```python
from build123d import *


with BuildPart() as part:
    # 扫描1: sweep along a path in 草图1
    with BuildLine(Plane(origin=(0, 0, 0), x_dir=(0, 0, -1), z_dir=(1, 0, 0))) as sweep_1_path:
        Line((9.103840683, 79.480312561), (356.051920341, 39.740156281))
        ThreePointArc((356.051920341, 39.740156281), (391.5, 0), (356.051920341, -39.740156281))
        Line((356.051920341, -39.740156281), (9.103840683, -79.480312561))
        ThreePointArc((9.103840683, -79.480312561), (-80, 0), (9.103840683, 79.480312561))
    # 草图2 → 扫描1 (sweep)
    with BuildSketch(Plane.XY):
        Polygon((-5, 80), (5, 80), (3.165615911, 74), (-3.165615911, 74), align=None)
    sweep(path=sweep_1_path.line)


solid = part.part
```
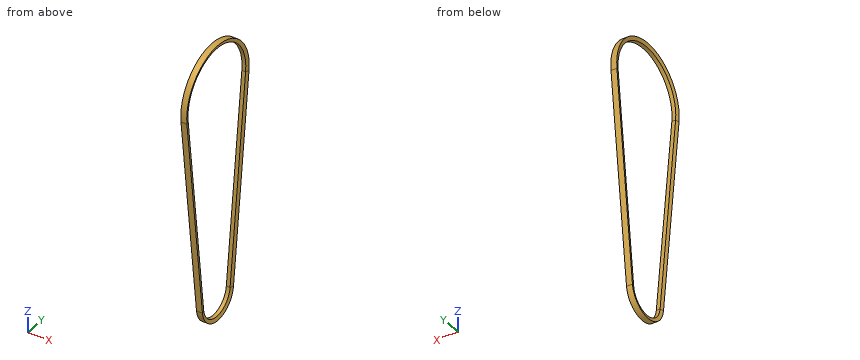
The model under review builds one solid part; all positions refer to its coordinate system, in mm. Coordinates: 2 decimals unless noted, no trailing zeros. Write each loop counter-clockwise with the first axis right and the second up, starting at its lowest first coordinate (ties: lowest second). Pieces come first, ordered by that corner, then holes. Notation, with made-up numbers: (16.5, 42) - (44.5, 42) arc R5 cw to (44.5, 48) - close; hole circle Ø5 at (57, 4). An arc over 180 degrees is marked (long way). Answer in a Markdown table with one row per item. Add a question column.
Q1. Consider section B-B on y = 0. Give the boundary of the cut face in (x, z), then the cut area to 3 significant figures.
Q2. Consider section C-C on x = 0.75. Give the boundary of the cut face in (y, z).
Q3. Clearance check with flat-ended pins moving along their axes: pin 1 (2 mm diameter, centred on x = 1, y = -33.5, fed in from -Z); pin 2 (12 mm diameter, centred on y = 47, z = -304, fed in from +X); pin 3 (1 mm diameter, centred on x = -1, y = 43.5, fed in from +Z). State where each tip first meets the part, or that it passes through.
Q4. Consider section A-A on z = 0. Give the boundary of the cut face in (x, y), then the cut area to 3 significant figures.
Q5. To check wall thickness, follow line 1 along Y through (x, z) = (-0.5, 0); line 2 along Z through (x, y) = (1.75, 0); line 3 along Y through (x, z) = (0.75, 30). State the ranges of each line that lie inside material, in increasing order. Write a range as from..to.
Answers below:
| question | item | result |
|---|---|---|
| 1 | outline | (-5, -391.5) - (5, -391.5) - (3.17, -385.5) - (-3.17, -385.5) - close; (-5, 80) - (-3.17, 74) - (3.17, 74) - (5, 80) - close |
| 1 | area | 98.0 mm² |
| 2 | outline | (-79.48, -9.1) - (-39.74, -356.05) arc R40 ccw to (39.74, -356.05) - (79.48, -9.1) arc R80 ccw (long way) to start; hole (-73.52, -8.42) - (-33.78, -355.37) arc R34 ccw to (33.78, -355.37) - (73.52, -8.42) arc R74 ccw (long way) to start |
| 3 | pin 1 | z = -374.82 |
| 3 | pin 2 | x = 5 |
| 3 | pin 3 | z = 67.46 |
| 4 | outline | (-5, -80) - (5, -80) - (3.17, -74) - (-3.17, -74) - close; (-5, 80) - (-3.17, 74) - (3.17, 74) - (5, 80) - close |
| 4 | area | 98.0 mm² |
| 5 | line 1 | -80..-74, 74..80 |
| 5 | line 2 | -391.5..-385.5, 74..80 |
| 5 | line 3 | -74.16..-67.65, 67.65..74.16 |
